Geometry: final body of the model. Coordinates: model frame, mm. Give positions to 0.01 mm unless a question says otherwise; leave off trailing zeros. Loops run counter-clockwise (first coordinate to the right, second up) from the corner with the lowest first, then second, coordinate; pieces in that order, holes last. Notation, with made-up numbers: (-30.5, 71.25) - (-6.5, 71.25) arc R34 ccw to (-6.5, 103.25) - close; hole circle Ø5 at (36.25, 76.5). An arc over 180 degrees is marked (long way). Use one line per item in the form item = value.
```python
from build123d import *

# Parameters (mm, degrees)
SKETCH1_W            = 535
SKETCH1_H            = 230
BOSS_EXTRUDE1_DEPTH  = 2.5
FILLET1_R            = 10
SKETCH2_R            = 3.5
CUT_EXTRUDE1_DEPTH   = 2.5
LPATTERN1_COUNT      = 2
LPATTERN1_PITCH      = 515
LPATTERN1_COUNT_DIR2 = 2
LPATTERN1_PITCH_DIR2 = 210
SKETCH3_W            = 124
SKETCH3_H            = 111
CUT_EXTRUDE2_DEPTH   = 2.5
SKETCH4_W            = 234
SKETCH4_H            = 48.5
CUT_EXTRUDE3_DEPTH   = 2.5
SKETCH5_R            = 11.5
CUT_EXTRUDE4_DEPTH   = 2.5
SKETCH7_R            = 8.25
CUT_EXTRUDE5_DEPTH   = 2.5
SKETCH8_W            = 54
SKETCH8_H            = 183
CUT_EXTRUDE6_DEPTH   = 2.5


with BuildPart() as part:
    # Sketch1 → Boss-Extrude1 (new body)
    with BuildSketch(Plane.XY):
        with Locations((267.5, -115)):
            Rectangle(SKETCH1_W, SKETCH1_H)
    extrude(amount=BOSS_EXTRUDE1_DEPTH)

    # Fillet1
    fillet1_edges = [part.edges().sort_by_distance(p)[0] for p in [
        (0, 0, 1.25),
        (535, 0, 1.25),
        (535, -230, 1.25),
        (0, -230, 1.25),
    ]]
    fillet(fillet1_edges, radius=FILLET1_R)

    # Sketch2 → Cut-Extrude1 (cut)
    with BuildSketch(Plane.XY.offset(2.5)):
        with Locations((10, -10)):
            Circle(SKETCH2_R)
    cut_extrude1 = extrude(amount=-CUT_EXTRUDE1_DEPTH, mode=Mode.SUBTRACT)

    # LPattern1: Cut-Extrude1 2 × 2
    with Locations(*[(i * LPATTERN1_PITCH, -j * LPATTERN1_PITCH_DIR2, 0) for i in range(LPATTERN1_COUNT) for j in range(LPATTERN1_COUNT_DIR2) if (i, j) != (0, 0)]):
        add(cut_extrude1, mode=Mode.SUBTRACT)

    # Sketch3 → Cut-Extrude2 (cut)
    with BuildSketch(Plane.XY.offset(2.5)):
        with Locations((104, -76.5)):
            Rectangle(SKETCH3_W, SKETCH3_H)
    extrude(amount=-CUT_EXTRUDE2_DEPTH, mode=Mode.SUBTRACT)

    # Sketch4 → Cut-Extrude3 (cut)
    with BuildSketch(Plane.XY.offset(2.5)):
        with Locations((183, -180.75)):
            Rectangle(SKETCH4_W, SKETCH4_H)
    extrude(amount=-CUT_EXTRUDE3_DEPTH, mode=Mode.SUBTRACT)

    # Sketch5 → Cut-Extrude4 (cut)
    with BuildSketch(Plane.XY.offset(2.5)):
        with Locations((36, -188)):
            Circle(SKETCH5_R)
    extrude(amount=-CUT_EXTRUDE4_DEPTH, mode=Mode.SUBTRACT)

    # Sketch7 → Cut-Extrude5 (cut)
    with BuildSketch(Plane.XY.offset(2.5)):
        with Locations((36, -152)):
            Circle(SKETCH7_R)
    extrude(amount=-CUT_EXTRUDE5_DEPTH, mode=Mode.SUBTRACT)

    # Sketch8 → Cut-Extrude6 (cut)
    with BuildSketch(Plane.XY.offset(2.5)):
        with Locations((473, -115)):
            Rectangle(SKETCH8_W, SKETCH8_H)
    extrude(amount=-CUT_EXTRUDE6_DEPTH, mode=Mode.SUBTRACT)


solid = part.part
```
(1) Cut plane A-A (x = 36). Return the cut outline in (y, z).
Solution:
outline = (-230, 0) - (-199.5, 0) - (-199.5, 2.5) - (-230, 2.5) - close; (-176.5, 0) - (-160.25, 0) - (-160.25, 2.5) - (-176.5, 2.5) - close; (-143.75, 0) - (0, 0) - (0, 2.5) - (-143.75, 2.5) - close
(2) Pull-direction query (X, two-part tool) for faces 1 (the face through (2.85, -3.01, 1.27)), 2 (the face through (323, -113, 0)), 3 (the face through (34.93, -143.82, 1.27)); classes: released by +X, released by -X, zero draft, split by the parting line, or undercut.
Solution:
face_1 = released by -X
face_2 = zero draft
face_3 = undercut
(3) Pin query (flat end, axial travel): P1, Ø4, axis at x = 10, y = -10, coming from the +Z side. Return the tip coordinate at first contact, or that it passes through.
Solution:
P1 = through
(4) Material intervals for L1, parallel to X at y = -119.5, z = 0.5; L2, parallel to X at y = -166.5, z = 2.15; L3, parallel to Y at x = 10, z = 1.3, sorted ascending. Write a range as from..to.
Solution:
L1 = 0..42, 166..446, 500..535
L2 = 0..66, 300..446, 500..535
L3 = -230..-223.5, -216.5..-13.5, -6.5..0
(5) Cut plane B-B (y = -188). Return the cut outline in (x, z), plus the area to 3 significant figures.
Solution:
outline = (0, 0) - (24.5, 0) - (24.5, 2.5) - (0, 2.5) - close; (47.5, 0) - (66, 0) - (66, 2.5) - (47.5, 2.5) - close; (300, 0) - (446, 0) - (446, 2.5) - (300, 2.5) - close; (500, 0) - (535, 0) - (535, 2.5) - (500, 2.5) - close
area = 560 mm2
(6) Cut plane D-D (x = 202.5). Return the cut outline in (y, z).
Solution:
outline = (-230, 0) - (-205, 0) - (-205, 2.5) - (-230, 2.5) - close; (-156.5, 0) - (0, 0) - (0, 2.5) - (-156.5, 2.5) - close
(7) Cut plane C-C (z = 1.3). Give the number of separate pieces and of enclosed holes in the cut face, plus the area to 3 significant figures.
Solution:
separate_pieces = 1
enclosed_holes = 9
area = 87,200 mm2
